Source: three-view drawing plus pictorial views. Frame: mm from the lowest corner of the part. Round coordinates to 2 decimals unless told otherwise and drop trailing zeros. Loops run counter-clockwise (first coordinate to the right, second up) from the corner with the lowest first, then second, coordinate; pieces in that order, holes last. Notation, with made-up numbers: (37, -1) -> (90, -1) arc R21 ccw to (90, 20) -> close; hole circle Ø8 at (37, 44.5). An arc over 180 degrees is marked (long way). Answer in a Markdown table with one row per item.
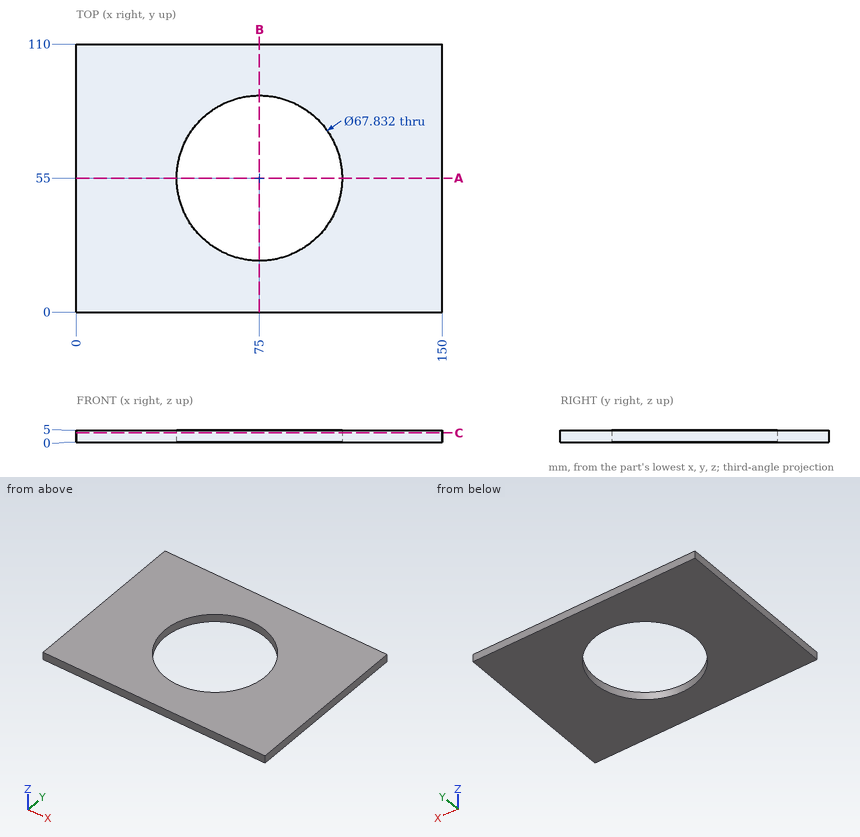
Item 1: Cut plane C-C (z = 3.9). Output: boundary loops of the cut face in (x, y), then the cut area to 3 significant figures.
Answer:
| item | result |
|---|---|
| outline | (0, 0) -> (150, 0) -> (150, 110) -> (0, 110) -> close; hole circle Ø67.83 at (75, 55) |
| area | 12,900 mm² |
Item 2: Line query: probe 1 along Y at (x, z) = (75, 3.4); probe 2 along X at (y, z) = (65, 3.05); probe 3 along Y at (x, z) = (68.5, 3.95). Output: solid intervals per line, ascending. Write a range as [from, to].
Answer:
| item | result |
|---|---|
| probe 1 | y = [0, 21.08], [88.92, 110] |
| probe 2 | x = [0, 42.59], [107.41, 150] |
| probe 3 | y = [0, 21.71], [88.29, 110] |
Item 3: Cut plane B-B (x = 75). Output: boundary loops of the cut face in (y, z), then the cut area to 3 significant figures.
Answer:
| item | result |
|---|---|
| outline | (0, 0) -> (21.08, 0) -> (21.08, 5) -> (0, 5) -> close; (88.92, 0) -> (110, 0) -> (110, 5) -> (88.92, 5) -> close |
| area | 211 mm² |
Item 4: Cut plane A-A (y = 55). Output: boundary loops of the cut face in (x, z), then the cut area to 3 significant figures.
Answer:
| item | result |
|---|---|
| outline | (0, 0) -> (41.08, 0) -> (41.08, 5) -> (0, 5) -> close; (108.92, 0) -> (150, 0) -> (150, 5) -> (108.92, 5) -> close |
| area | 411 mm² |
